```python
from build123d import *

# Parameters (mm, degrees)
SKETCH_1_W                  = 12
SKETCH_1_H                  = 68
EXTRUDE_1_DEPTH             = 33
HOLE_WIZARD_M6_1_D          = 5
HOLE_WIZARD_M6_1_DEPTH      = 15
HOLE_WIZARD_M6_1_TIP        = 1.502151548
HOLE_WIZARD_M5_1_D          = 4.2
HOLE_WIZARD_M5_1_DEPTH      = 11
HOLE_WIZARD_M5_1_TIP        = 1.2618073
HOLE_WIZARD_C_0_D           = 5.5
HOLE_WIZARD_C_0_CBORE_D     = 10
HOLE_WIZARD_C_0_CBORE_DEPTH = 5.5
CHAMFER_1_SIZE              = 1


with BuildPart() as part:
    # 草图1 → 凸台-拉伸1 (new body)
    with BuildSketch(Plane.XY):
        with Locations((-70.482202682, -45.607833778)):
            Rectangle(SKETCH_1_W, SKETCH_1_H)
    extrude(amount=-EXTRUDE_1_DEPTH)

    # M6 螺纹孔1
    with Locations(Plane.ZY.offset(76.482202682)):
        with Locations((-16.5, -73.607833778), (-8, -49.607833778), (-25, -49.607833778)):
            Hole(HOLE_WIZARD_M6_1_D / 2, depth=HOLE_WIZARD_M6_1_DEPTH)
            with Locations((0, 0, -(HOLE_WIZARD_M6_1_DEPTH + HOLE_WIZARD_M6_1_TIP / 2))):  # 118° drill point
                Cone(0, HOLE_WIZARD_M6_1_D / 2, HOLE_WIZARD_M6_1_TIP, mode=Mode.SUBTRACT)

    # M5 螺纹孔1
    with Locations(Plane(origin=(0, -11.607833778, 0), x_dir=(1, 0, 0), z_dir=(0, 1, 0))):
        with Locations((-70.482202682, 26), (-70.482202682, 7)):
            Hole(HOLE_WIZARD_M5_1_D / 2, depth=HOLE_WIZARD_M5_1_DEPTH)
            with Locations((0, 0, -(HOLE_WIZARD_M5_1_DEPTH + HOLE_WIZARD_M5_1_TIP / 2))):  # 118° drill point
                Cone(0, HOLE_WIZARD_M5_1_D / 2, HOLE_WIZARD_M5_1_TIP, mode=Mode.SUBTRACT)

    # 打孔尺寸根据六角头螺栓 C 级的类型0 (through all)
    with Locations(Plane.ZY.offset(76.482202682)):
        with Locations((-16.5, -19.604255019), (-16.5, -39.607833778)):
            CounterBoreHole(HOLE_WIZARD_C_0_D / 2, HOLE_WIZARD_C_0_CBORE_D / 2, HOLE_WIZARD_C_0_CBORE_DEPTH)

    # 倒角1
    chamfer_1_edges = [part.edges().sort_by_distance(p)[0] for p in [
        (-70.482202682, -11.607833778, -33),
        (-70.482202682, -11.607833778, 0),
        (-70.482202682, -79.607833778, 0),
        (-70.482202682, -79.607833778, -33),
    ]]
    chamfer(chamfer_1_edges, length=CHAMFER_1_SIZE)


solid = part.part
```
CAD build for the part. Positions are in the model's coordinates, mm. A direction names the side the tool comes from. Round coordinates to 2 decimals unless told otherwise and drop trailing zeros. Order: outer loops, then holes, each group sorted by start corner. A loop starts at its lowest first (then second) coordinate and runs counter-clockwise, first axis right, second up. Notation, with made-up numbers: (89.5, 57) - (96.5, 57) arc R17 cw to (96.5, 69) - close; hole circle Ø1 at (34, 36). An arc over 180 degrees is marked (long way). Use CSV: the item, a comma, the result in double quotes. Start each with the question number.
1) Pin check, flat tips, straight feed: pin 1 Ø13 at (y, z) = (-39.61, -16.5) entering from +X; pin 2 Ø3.5 at (x, z) = (-70.48, -7) entering from +Y; pin 3 Ø5 at (y, z) = (-19, -18) entering from -X. Stop position of each tip, or through.
2) Tool access for faces 1 (the cylindrical face through (-68.384, -17.185, -7.092)), 2 (the flat face through (-70.982, -22, -14)), 3 (the flat face through (-71, -11.608, -16)): list every direction of +Z, -Z, +X, -X, +Y, -Y with a clear straight run to the whole face (end or side of a thin tool).
3) Wall check: L1, parallel to Y at x = -72.4, z = -16.5; L2, parallel to Y at x = -73, z = -25; L3, parallel to Z at x = -67.5, y = -19.5. Give the ranges that are in metal, low to high. Write a range as [from, to].
4) Saw through at B-B (x = -65.25). List the corners of the cut face in (y, z), and give its area (3 significant figures).
5) Two-plate mould, pull along Y, no slides. Class faces 4 (the flat face through (-64.482, -46, -16)), 5 (the conical face through (-70.75, -23.65, -26.25)), 6 (the cylindrical face through (-73.77, -34.65, -17.15)): pulls with the +Y half, pulls with the -Y half, needs draft (parallel to the pull), parting line crosses it, or undercut.
6) Saw through at A-A (y = -41). List the corners of the cut face in (x, z).
Values follow:
1,pin 1,"stops at x = -64.48"
1,pin 2,"stops at y = -22.82"
1,pin 3,"stops at x = -70.98"
2,face 1,"+Y"
2,face 2,"-X"
2,face 3,"+Z, -Z, +X, -X, +Y"
3,L1,"y = [-79.61, -76.11], [-71.11, -44.61], [-34.61, -24.6], [-14.6, -11.61]"
3,L2,"y = [-79.61, -52.11], [-47.11, -11.61]"
3,L3,"z = [-33, -19.25], [-13.75, 0]"
4,outline,"(-79.61, -32) - (-78.61, -33) - (-12.61, -33) - (-11.61, -32) - (-11.61, -1) - (-12.61, 0) - (-78.61, 0) - (-79.61, -1) - close; hole circle Ø5 at (-73.61, -16.5); hole circle Ø5 at (-49.61, -25); hole circle Ø5 at (-49.61, -8); hole circle Ø5.5 at (-39.61, -16.5); hole circle Ø5.5 at (-19.6, -16.5)"
4,area,"2,140 mm2"
5,face 4,"needs draft"
5,face 5,"pulls with the +Y half"
5,face 6,"undercut"
6,outline,"(-76.48, -33) - (-64.48, -33) - (-64.48, -18.87) - (-70.98, -18.87) - (-70.98, -21.3) - (-76.48, -21.3) - close; (-76.48, -11.7) - (-70.98, -11.7) - (-70.98, -14.13) - (-64.48, -14.13) - (-64.48, 0) - (-76.48, 0) - close"
